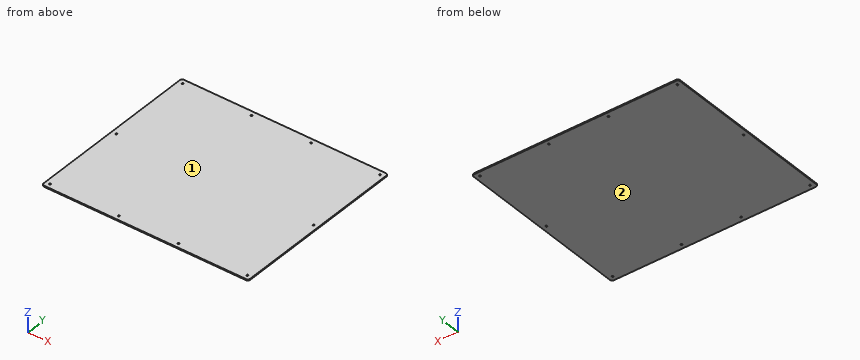
from build123d import *

# Parameters (mm, degrees)
SKETCH_1_W                = 900
SKETCH_1_H                = 780
EXTRUDE_1_DEPTH           = 5
HOLE_WIZARD_7_0_7_1_D     = 7
HOLE_WIZARD_7_0_7_1_DEPTH = 27.75
HOLE_WIZARD_7_0_7_1_TIP   = 2.103012167
FILLET_1_R                = 10


with BuildPart() as part:
    # 草图1 → 凸台-拉伸1 (new body)
    with BuildSketch(Plane.XY):
        Rectangle(SKETCH_1_W, SKETCH_1_H)
    extrude(amount=EXTRUDE_1_DEPTH)

    # Ø7.0 (7) 直径孔1
    with Locations(Plane.XY.offset(5)):
        with Locations((-430, 370), (430, 370), (430, -370), (-430, -370), (-430, 0), (430, 0), (-130, 370), (130, 370), (-130, -370), (130, -370)):
            Hole(HOLE_WIZARD_7_0_7_1_D / 2, depth=HOLE_WIZARD_7_0_7_1_DEPTH)
            with Locations((0, 0, -(HOLE_WIZARD_7_0_7_1_DEPTH + HOLE_WIZARD_7_0_7_1_TIP / 2))):  # 118° drill point
                Cone(0, HOLE_WIZARD_7_0_7_1_D / 2, HOLE_WIZARD_7_0_7_1_TIP, mode=Mode.SUBTRACT)

    # 圆角1
    fillet_1_edges = [part.edges().sort_by_distance(p)[0] for p in [
        (450, -390, 2.5),
        (-450, -390, 2.5),
        (-450, 390, 2.5),
        (450, 390, 2.5),
    ]]
    fillet(fillet_1_edges, radius=FILLET_1_R)


solid = part.part
Design review of the part built by this model. Coordinates are the model's own, in mm. Face numbers are marked on the shaded views. Coordinates: 2 decimals unless noted, no trailing zeros. One line per item, written item: value.
1) To check wall thickness, follow probe 1 along X at (y, z) = (370, 3.05); probe 2 along Y at (x, z) = (430, 2); probe 3 along Y at (x, z) = (-130, 2.7). State the ranges of each line that lie inside material, in increasing order.
Answer sheet:
probe 1: x = -450 to -433.5, -426.5 to -133.5, -126.5 to 126.5, 133.5 to 426.5, 433.5 to 450
probe 2: y = -390 to -373.5, -366.5 to -3.5, 3.5 to 366.5, 373.5 to 390
probe 3: y = -390 to -373.5, -366.5 to 366.5, 373.5 to 390
2) Mouldability with a two-part tool opening along Z and no side actions: class the marked faces 1 and 2 as +Z half, -Z half, draft (parallel to the pull), parting line (faces both ways), or undercut.
Answer sheet:
face 1: +Z half
face 2: -Z half
3) Insertion check: pin 1 (6.5 mm diameter, centred on x = -130, y = 370, fed in from -Z). The pin has a flat end and moves straight along its axis. Give the tip position at first contact, or say it passes through.
Answer sheet:
pin 1: passes through
